Can you work these out from the drawing? Everything is in mm from the part's minimum corner. Give positions to 0.01 mm unless a question says otherwise; leave off trailing zeros. Order: outer loops, then holes, each group sorted by start corner. A loop starts at its lowest first (then second) coordinate and runs counter-clockwise, first axis right, second up. Notation, with made-up numbers: M 48,-38 L 69,-38 A10 cw 69,-21 Z; hole C -24,-18 d2. An arc over 180 degrees is marked long. Use a Markdown table: item, result. Add a question column.
Item 1: Suppose I cut it at A-A on y = 65. Write out the boundary of the cut face in (x, z), plus the area to 3 significant figures.
Item 2: Suppose I cut it at C-C on z = 10. Count the separate pieces of the cut face and the enclosed holes in it, plus the area to 3 significant figures.
Item 3: If I drill on L1, parallel to X at y = 285, z = 12.25; L2, parallel to X at y = 64, z = 10.5, over which ranges is the centre line in solid material (lowest first)? Write a range as from..to.
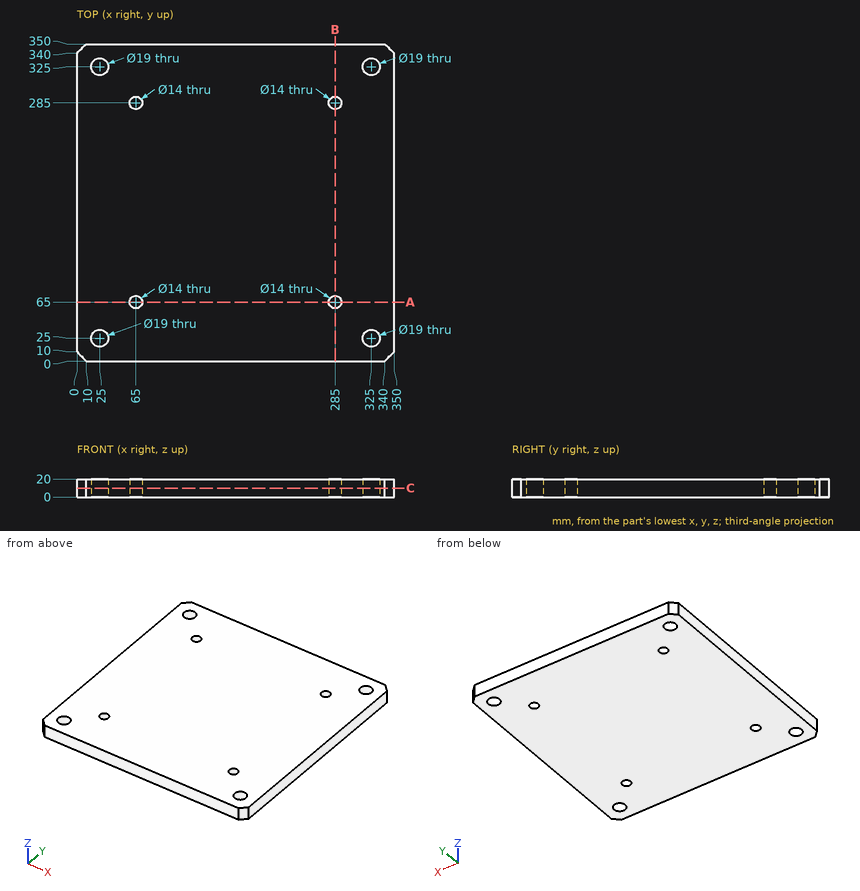
Findings below:
| question | item | result |
|---|---|---|
| 1 | outline | M 0,0 L 58,0 L 58,20 L 0,20 Z; M 72,0 L 278,0 L 278,20 L 72,20 Z; M 292,0 L 350,0 L 350,20 L 292,20 Z |
| 1 | area | 6,440 mm^2 |
| 2 | separate pieces | 1 |
| 2 | enclosed holes | 8 |
| 2 | area | 121,000 mm^2 |
| 3 | L1 | x = 0..58, 72..278, 292..350 |
| 3 | L2 | x = 0..58.07, 71.93..278.07, 291.93..350 |
